```python
from build123d import *

# Parameters (mm, degrees)
CHAMFER_1_SIZE = 0.5


with BuildPart() as part:
    # 草图1 → 旋转1 (revolve)
    with BuildSketch(Plane.XY, mode=Mode.PRIVATE) as revolve_1_sk:
        Polygon((0, 17.5), (21, 17.5), (21, 21.25), (26, 21.25), (26, 17.5), (29, 17.5), (29, 23), (0, 23), align=None)
    revolve(revolve_1_sk.sketch.rotate(Axis((0, 0, 0), (1, 0, 0)), 90), axis=Axis((0, 0, 0), (1, 0, 0)))

    # 倒角1
    chamfer_1_edges = [part.edges().sort_by_distance(p)[0] for p in [
        (29, 0, -23),
        (0, 0, -23),
    ]]
    chamfer(chamfer_1_edges, length=CHAMFER_1_SIZE)


solid = part.part
```
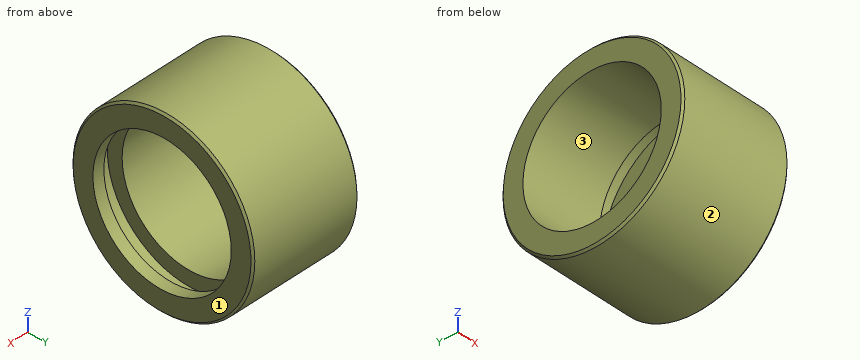
Could you check a few things on this model? Use its own coordinates, in mm. Face numbers are marked on the shaded views. Coordinates: 2 decimals unless noted, no trailing zeros. Order: outer loops, then holes, each group sorted by start corner. A loop starts at its lowest first (then second) coordinate and runs counter-clockwise, first axis right, second up. Notation, with made-up numbers: M -38,87 L -25,87 A19 ccw -25,119 Z; hole C -29.5,61 d5. An arc over 180 degrees is marked long. Use one line per item in the form item = value. Start each with the question number.
1. Suppose I cut it at C-C on x = 12.25. Write out the boundary of the cut face in (y, z).
2. Please list where these lines run through material, in increasing order: line 1 (X direction, y = 8, z = 16); line 2 (Y direction, x = 26.85, z = 0); line 3 (Y direction, x = 13, z = 13.5).
3. For pin 1 (10 mm diameter, centred on x = 9, z = -12, fed in from -Y); pin 2 (3 mm diameter, centred on x = 12.5, y = 9, fed in from +Z); pin 3 (8 mm diameter, centred on x = 13.5, z = -7.5, fed in from +Y), each with a flat end and sliding along its axis, tell me the tip position at first contact or that it passes through.
4. Suppose I cut it at A-A on z = 0. Write out the boundary of the cut face in (x, y), then the cut area to 3 significant figures.
5. We'd pull the mould along Z, two halves only. Please class the marked faces 1, 2 and 3: +Z half, -Z half, draft (parallel to the pull), parting line (faces both ways), or undercut.
Geometry says:
q1.outline = C 0,0 d46; hole C 0,0 d35
q2.line_1 = 0 to 21, 26 to 29
q2.line_2 = -23 to -17.5, 17.5 to 23
q2.line_3 = -18.62 to -11.14, 11.14 to 18.62
q3.pin_1 = -21.91
q3.pin_2 = 21.74
q3.pin_3 = 22.73
q4.outline = M 0,-22.5 L 0.5,-23 L 28.5,-23 L 29,-22.5 L 29,-17.5 L 26,-17.5 L 26,-21.25 L 21,-21.25 L 21,-17.5 L 0,-17.5 Z; M 0,17.5 L 21,17.5 L 21,21.25 L 26,21.25 L 26,17.5 L 29,17.5 L 29,22.5 L 28.5,23 L 0.5,23 L 0,22.5 Z
q4.area = 281 mm^2
q5.face_1 = draft
q5.face_2 = parting line
q5.face_3 = undercut
